Answer from the drawing. Dimensions are ordinates in mm from the lowest x, y and z of the part. Give positions to 0.01 mm unless a question says otherwise; leave off trailing zeros. Write each loop counter-clockwise with the first axis right and the second up, starting at its lowest first coordinate (ties: lowest second). Pieces come first, ordered by that corner, then holes.
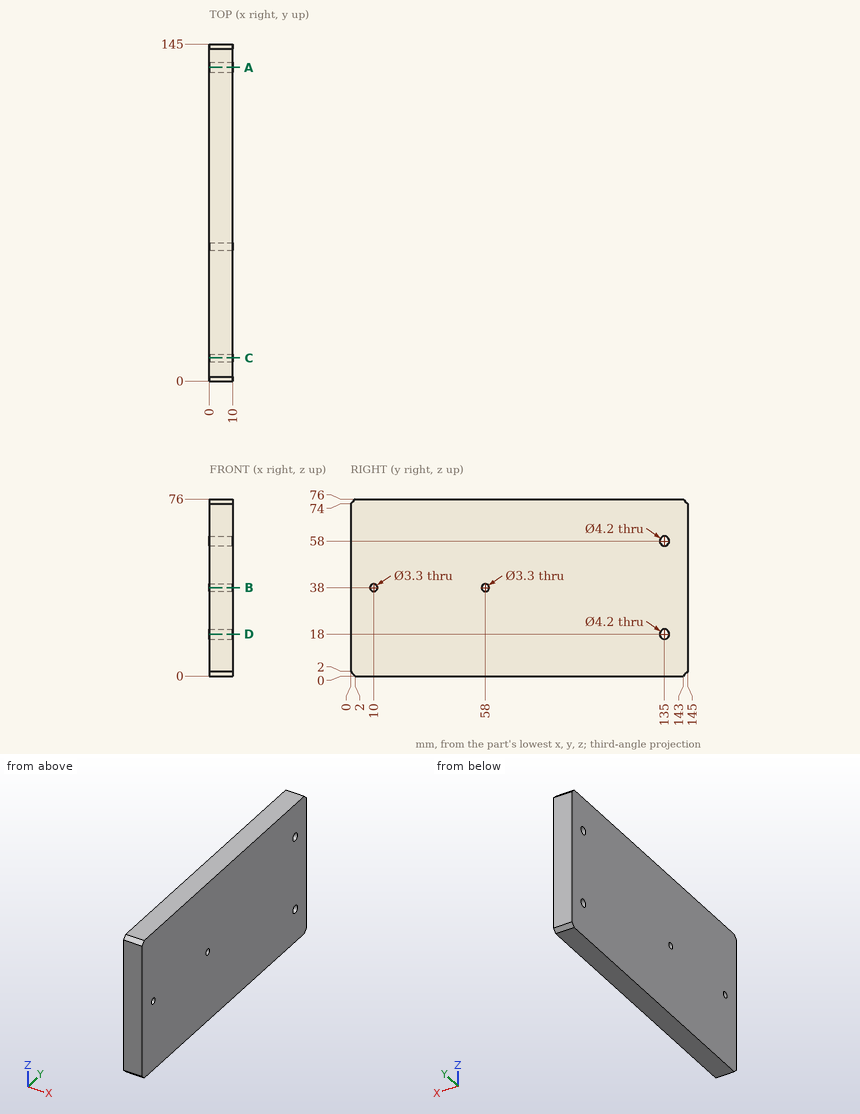
Item 1: This flat-tipped pin is pushed along its axis until it touches: P1, Ø6.5, axis at y = 135, z = 58, coming from the -X side. Where does it stop, or does it pass through?
Conclusion:
P1: stops at x = 0
Item 2: A cutting plane is placed at C-C, the plane y = 10. Give the vertices of the cut face in (x, z).
Conclusion:
outline: (0, 0) - (10, 0) - (10, 36.35) - (0, 36.35) - close; (0, 39.65) - (10, 39.65) - (10, 76) - (0, 76) - close
Item 3: A cutting plane is placed at A-A, the plane y = 135. Give the vertices of the cut face in (x, z).
Conclusion:
outline: (0, 0) - (10, 0) - (10, 15.9) - (0, 15.9) - close; (0, 20.1) - (10, 20.1) - (10, 55.9) - (0, 55.9) - close; (0, 60.1) - (10, 60.1) - (10, 76) - (0, 76) - close
Item 4: A cutting plane is placed at B-B, the plane z = 38. Give the vertices of the cut face in (x, y), plus the area to 3 significant figures.
Conclusion:
outline: (0, 0) - (10, 0) - (10, 8.35) - (0, 8.35) - close; (0, 11.65) - (10, 11.65) - (10, 56.35) - (0, 56.35) - close; (0, 59.65) - (10, 59.65) - (10, 145) - (0, 145) - close
area: 1,380 mm2
Item 5: Consider probe 1 along Y at (x, z) = (7.5, 38); probe 2 along Z at (x, y) = (3.5, 135); probe 3 along Y at (x, z) = (3.5, 18). Determine where each line is inside the solid, lowest interval first.
Conclusion:
probe 1: y = 0 to 8.35, 11.65 to 56.35, 59.65 to 145
probe 2: z = 0 to 15.9, 20.1 to 55.9, 60.1 to 76
probe 3: y = 0 to 132.9, 137.1 to 145
Item 6: A cutting plane is placed at D-D, the plane z = 18. Give the vertices of the cut face in (x, y).
Conclusion:
outline: (0, 0) - (10, 0) - (10, 132.9) - (0, 132.9) - close; (0, 137.1) - (10, 137.1) - (10, 145) - (0, 145) - close
